from build123d import *

# Parameters (mm, degrees)
BASE_PLATE_SKETCH_W     = 99
BASE_PLATE_SKETCH_H     = 50
BASE_PLATE_DEPTH        = 10
SUPPORT_BLOCK_SKETCH_W  = 99
SUPPORT_BLOCK_SKETCH_H  = 15
SUPPORT_BLOCK_DEPTH     = 40
SUPPORT_TAPER_CUT_DEPTH = 40
CYLINDER_BOSS_SKETCH_R  = 20
CYLINDER_BOSS_40_DEPTH  = 25
END_SLOT_SKETCH_W       = 47.327731092
END_SLOT_SKETCH_H       = 16
END_SLOT_16X8_DEPTH     = 8


with BuildPart() as part:
    # Base Plate Sketch → Base Plate (new body)
    with BuildSketch(Plane(origin=(0, 0, 0), x_dir=(1, 0, 0), z_dir=(0, 1, 0))):
        Rectangle(BASE_PLATE_SKETCH_W, BASE_PLATE_SKETCH_H)
    extrude(amount=BASE_PLATE_DEPTH)

    # Support Block Sketch → Support Block (add)
    with BuildSketch(Plane(origin=(0, 10, 0), x_dir=(1, 0, 0), z_dir=(0, 1, 0))):
        Rectangle(SUPPORT_BLOCK_SKETCH_W, SUPPORT_BLOCK_SKETCH_H)
    extrude(amount=SUPPORT_BLOCK_DEPTH)

    # Support Taper Sketch → Support Taper Cut (cut, symmetric)
    with BuildSketch(Plane.XY):
        Polygon((-25, 50), (-49.5, 0), (-49.5, 50), align=None)
        Polygon((25, 50), (49.5, 0), (49.5, 50), align=None)
    extrude(amount=SUPPORT_TAPER_CUT_DEPTH, both=True, mode=Mode.SUBTRACT)

    # Cylinder Boss Sketch → Cylinder Boss Ø40 (add, symmetric)
    with BuildSketch(Plane.XY):
        with Locations((0, 40)):
            Circle(CYLINDER_BOSS_SKETCH_R)
    extrude(amount=CYLINDER_BOSS_40_DEPTH, both=True)

    # End Slot Sketch → End Slot 16x8 (cut)
    with BuildSketch(Plane.XY.offset(25)):
        with Locations((0, 40)):
            Rectangle(END_SLOT_SKETCH_W, END_SLOT_SKETCH_H)
    extrude(amount=-END_SLOT_16X8_DEPTH, mode=Mode.SUBTRACT)


solid = part.part
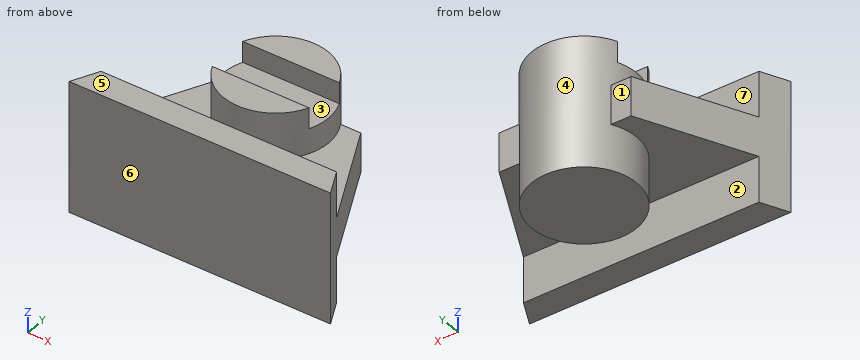
Here's how the part is built. I have some questions about the finished solid (model axes, mm). Face numbers are marked on the shaded views. A direction names the side the tool comes from. Round coordinates to 2 decimals unless told otherwise and drop trailing zeros. Write each loop counter-clockwise with the first axis right and the second up, starting at its lowest first coordinate (ties: lowest second). Pieces come first, ordered by that corner, then holes.
1. Will these pins go through, and if not, where does the flat tip stop? pin 1 Ø5 at (x, z) = (6, -19) entering from +Y; pin 2 Ø12 at (y, z) = (9, 16) entering from +X; pin 3 Ø2 at (x, y) = (-2, 18) entering from +Z.
2. Suppose I cut it at C-C (y = 40). List the corners of the cut face in (x, z) for me, and give its area (3 significant figures).
3. Suppose I cut it at D-D (z = -3.5). List the corners of the cut face in (x, y) for me.
4. Suppose I cut it at B-B (x = 0). List the corners of the cut face in (y, z) for me, and give its area (3 significant figures).
5. If we mould it in two halves opening along Y, with no side actions, what happens to the marked faces 5, 6 and 7? For each: released by +Y, released by -Y, zero draft, split by the parting line, or undercut.
6. For the marked faces 1, 2, 3 and 4, which set-ups out of +Z, -Z, +X, -X, +Y, -Y let a thin tool reach every point of the face, with its end or its side?
7. Suppose I cut it at A-A (z = -13). List the corners of the cut face in (x, y) for me.
8. I need wall thicknesses on L1, parallel to Z at x = -28, y = 33.5; L2, parallel to X at y = 40, z = 10; L3, parallel to Z at x = -8.5, y = 35. Which ranges of each line are inside material? Lowest first, please.
Answer sheet:
1. pin 1: stops at y = 59.69
1. pin 2: stops at x = 48.03
1. pin 3: stops at z = 7.5
2. outline: (-29.9, -7.5) - (-20, -7.5) - (-20, -25) - (20, -25) - (20, -7.5) - (29.9, -7.5) - (29.9, 7.5) - (20, 7.5) - (20, 17) - (-20, 17) - (-20, 7.5) - (-29.9, 7.5) - close
2. area: 1,980 mm2
3. outline: (-49.5, 0) - (49.5, 0) - (25, 50) - (17.32, 50) arc R20 ccw to (-17.32, 50) - (-25, 50) - close
4. outline: (0, -25) - (10, -25) - (10, -7.5) - (20, -7.5) - (20, -25) - (60, -25) - (60, 25) - (48, 25) - (48, 17) - (32, 17) - (32, 25) - (20, 25) - (20, 7.5) - (10, 7.5) - (10, 25) - (0, 25) - close
4. area: 2,520 mm2
5. face 5: zero draft
5. face 6: released by -Y
5. face 7: undercut
6. face 1: +Z, -Z, -X, +Y
6. face 2: -Z, +X, -X
6. face 3: +Z, +X, -X
6. face 4: none
7. outline: (-49.5, 0) - (49.5, 0) - (44.6, 10) - (-44.6, 10) - close; circle Ø40 at (0, 40)
8. L1: z = -7.5 to 7.5
8. L2: x = -20 to 20
8. L3: z = -25 to 17
